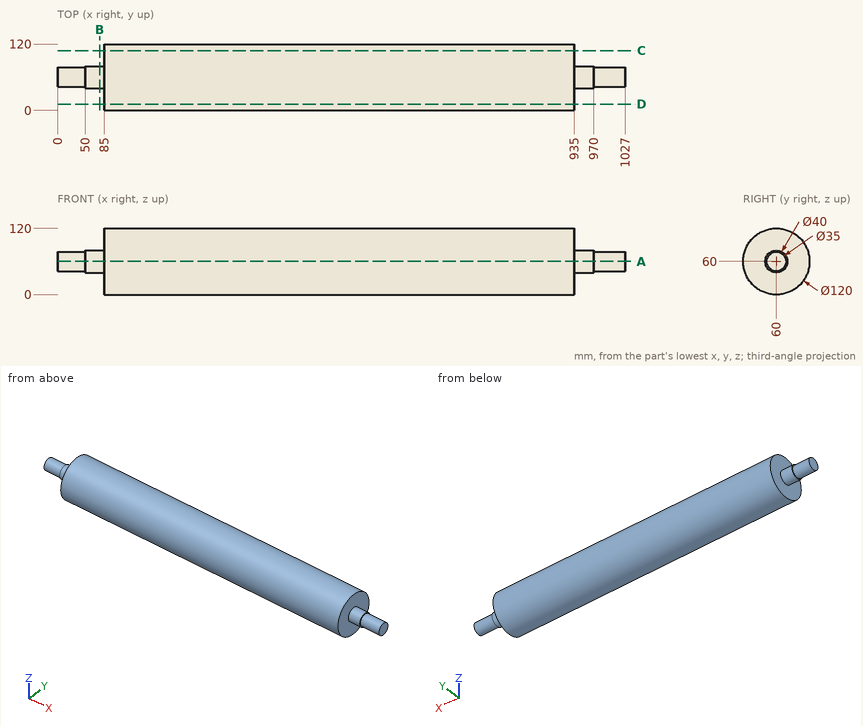
Here's the drawing with two shaded views (mm, measured from the low corner). I have some questions. Coordinates: 2 decimals unless noted, no trailing zeros. Order: outer loops, then holes, each group sorted by start corner. A loop starts at its lowest first (then second) coordinate and runs counter-clockwise, first axis right, second up.
Q1. Suppose I cut it at C-C on y = 108. Please give me the cut outline in (x, z), and give its area (3 significant figures).
Q2. Suppose I cut it at B-B on x = 76. Please give me the cut outline in (y, z), and give its area (3 significant figures).
Q3. Suppose I cut it at A-A on z = 60. Please give me the cut outline in (x, y), and give its area (3 significant figures).
Q4. Will these pins go through, and if not, where does the flat tip stop? pin 1 (1 mm diameter, centred on y = 36.5, z = 81, fed in from -X); pin 2 (5 mm diameter, centred on x = 507, z = 70, fed in from +Y); pin 3 (4 mm diameter, centred on x = 886.5, y = 43.5, fed in from +Z).
Q5. Please list where these lines run through material, in increasing order: L1, parallel to X at y = 22.5, z = 101.5; L2, parallel to Y at x = 474, z = 29.5; L3, parallel to Y at x = 169, z = 46.5.
Q6. Suppose I cut it at D-D on y = 11. Please give me the cut outline in (x, z).
Answer:
1. outline: (85, 24) - (935, 24) - (935, 96) - (85, 96) - close
1. area: 61,200 mm2
2. outline: circle Ø40 at (60, 60)
2. area: 1,260 mm2
3. outline: (0, 42.5) - (50, 42.5) - (50, 40) - (85, 40) - (85, 0) - (935, 0) - (935, 40) - (970, 40) - (970, 42.5) - (1027, 42.5) - (1027, 77.5) - (970, 77.5) - (970, 80) - (935, 80) - (935, 120) - (85, 120) - (85, 80) - (50, 80) - (50, 77.5) - (0, 77.5) - close
3. area: 109,000 mm2
4. pin 1: stops at x = 85
4. pin 2: stops at y = 119.53
4. pin 3: stops at z = 118.22
5. L1: x = 85 to 935
5. L2: y = 8.33 to 111.67
5. L3: y = 1.54 to 118.46
6. outline: (85, 25.37) - (935, 25.37) - (935, 94.63) - (85, 94.63) - close
